```python
from build123d import *

# Parameters (mm, degrees)
SKETCH1_R                      = 40
BOSS_EXTRUDE1_DEPTH            = 20
SKETCH2_R                      = 21
CUT_EXTRUDE1_DEPTH             = 11
SKETCH3_R                      = 18
CUT_EXTRUDE2_DEPTH             = 11
CUT_EXTRUDE3_DEPTH             = 61
M6_CLEARANCE_HOLE2_D           = 6.6
M6_CLEARANCE_HOLE2_CSINK_D     = 6.65
M6_CLEARANCE_HOLE2_CSINK_ANGLE = 90


with BuildPart() as part:
    # Sketch1 → Boss-Extrude1 (new body)
    with BuildSketch(Plane(origin=(0, 0, 0), x_dir=(1, 0, 0), z_dir=(0, 1, 0))):
        with Locations(Location((0, 0, 0), (0, 0, 270))):
            Circle(SKETCH1_R)
    extrude(amount=BOSS_EXTRUDE1_DEPTH)

    # Sketch2 → Cut-Extrude1 (cut)
    with BuildSketch(Plane(origin=(0, 20, 0), x_dir=(1, 0, 0), z_dir=(0, 1, 0))):
        with Locations(Location((0, 0, 0), (0, 0, 270))):
            Circle(SKETCH2_R)
    extrude(amount=-CUT_EXTRUDE1_DEPTH, mode=Mode.SUBTRACT)

    # Sketch3 → Cut-Extrude2 (cut)
    with BuildSketch(Plane(origin=(0, 9, 0), x_dir=(1, 0, 0), z_dir=(0, 1, 0))):
        with Locations(Location((0, 0, 0), (0, 0, 270))):
            Circle(SKETCH3_R)
    extrude(amount=-CUT_EXTRUDE2_DEPTH, mode=Mode.SUBTRACT)

    # Sketch8 → Cut-Extrude3 (cut, through all)
    with BuildSketch(Plane.XZ):
        with BuildLine():
            ThreePointArc((40, 0), (37.148351242, 14.832396974), (29, 27.549954628))
            Line((29, 27.549954628), (29, -27.549954628))
            ThreePointArc((29, -27.549954628), (37.148351242, -14.832396974), (40, 0))
        make_face()
        with BuildLine():
            ThreePointArc((-29, 27.549954628), (-40, 0), (-29, -27.549954628))
            Line((-29, -27.549954628), (-29, 27.549954628))
        make_face()
    extrude(amount=-CUT_EXTRUDE3_DEPTH, mode=Mode.SUBTRACT)

    # M6 Clearance Hole2 (through all)
    with Locations(Plane(origin=(0, 0, 0), x_dir=(-1, 0, 0), z_dir=(0, -1, 0))):
        with Locations((-15, -27.5), (15, -27.5), (15, 27.5), (-15, 27.5)):
            CounterSinkHole(M6_CLEARANCE_HOLE2_D / 2, M6_CLEARANCE_HOLE2_CSINK_D / 2, counter_sink_angle=M6_CLEARANCE_HOLE2_CSINK_ANGLE)


solid = part.part
```
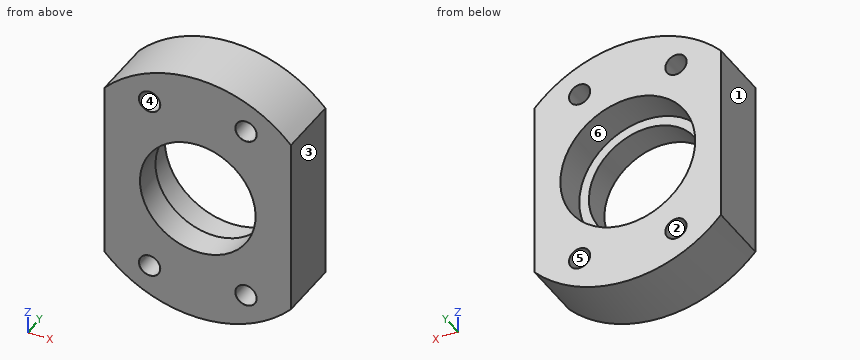
Source: CAD feature listing. Evaluate the final solid. Frame: model axes, mm. Face numbers are marked on the shaded views. A direction names the side the tool comes from. Round coordinates to 2 decimals unless told otherwise and drop trailing zeros. Order: outer loops, then holes, each group sorted by start corner. A loop starts at its lowest first (then second) coordinate and runs counter-clockwise, first axis right, second up. Notation, with made-up numbers: (77.25, 77.25) -> (86.25, 77.25) arc R24 ccw to (86.25, 92.25) -> close; hole circle Ø8 at (79, -26). An arc over 180 degrees is marked (long way). One line per item, written item: value. Start each with the question number.
Q1. Draft query along X for the marked faces 1, 2, 3 and 4. Return one class per face: pulls with the +X half, pulls with the -X half, needs draft (parallel to the pull), parting line crosses it, or undercut.
Q2. Section query C-C (y = 6.5). Return the cut outline in (x, z).
Q3. Pin query (flat end, axial travel): pin 1 (4 mm diameter, centred on x = -15, z = -27.5, fed in from +Y); pin 2 (6 mm diameter, centred on x = 17, z = 15, fed in from -Y); pin 3 (3 mm diameter, centred on x = -9.5, y = 16, fed in from -Z). Return the tip coordinate at first contact, or that it passes through.
Q4. Section query A-A (z = 0). Return the cut outline in (x, y).
Q5. Material intervals for probe 1 along X at (y, z) = (14.75, -27.5); probe 2 along Z at (x, y) = (16, 13.25); probe 3 along Z at (x, y) = (-13, 7.75), sorted ascending.
Q6. Access query for the marked faces 5 and 6. Directions: +Z, -Z, +X, -X, +Y, -Y. A direction counts if a zero-diameter tool reaches every point of the face in a straight line with its end or side. Return the directions, or none.
Q7. Section query B-B (x = 0). Return the cut outline in (y, z), plus the area to 3 significant figures.
Q8. Section query D-D (x = -15). Return the cut outline in (y, z) (3 decimals), plus the area to 3 significant figures.
Findings below:
1. face 1: pulls with the -X half
1. face 2: undercut
1. face 3: pulls with the +X half
1. face 4: undercut
2. outline: (-29, -27.55) arc R40 ccw to (29, -27.55) -> (29, 27.55) arc R40 ccw to (-29, 27.55) -> close; hole circle Ø6.6 at (-15, -27.5); hole circle Ø6.6 at (-15, 27.5); hole circle Ø36 at (0, 0); hole circle Ø6.6 at (15, -27.5); hole circle Ø6.6 at (15, 27.5)
3. pin 1: through
3. pin 2: y = 0
3. pin 3: z = -39.19
4. outline: (-29, 0) -> (-18, 0) -> (-18, 9) -> (-21, 9) -> (-21, 20) -> (-29, 20) -> close; (18, 0) -> (29, 0) -> (29, 20) -> (21, 20) -> (21, 9) -> (18, 9) -> close
5. probe 1: -29 to -18.3, -11.7 to 11.7, 18.3 to 29
5. probe 2: -36.66 to -30.64, -24.36 to -13.6, 13.6 to 24.36, 30.64 to 36.66
5. probe 3: -37.83 to -30.12, -24.88 to -12.45, 12.45 to 24.88, 30.12 to 37.83
6. face 5: +Y, -Y
6. face 6: +Y
7. outline: (0, -40) -> (20, -40) -> (20, -21) -> (9, -21) -> (9, -18) -> (0, -18) -> close; (0, 18) -> (9, 18) -> (9, 21) -> (20, 21) -> (20, 40) -> (0, 40) -> close
7. area: 814 mm²
8. outline: (0, -37.081) -> (20, -37.081) -> (20, -30.8) -> (0.025, -30.8) -> (0, -30.825) -> close; (0, -24.175) -> (0.025, -24.2) -> (20, -24.2) -> (20, -14.697) -> (9, -14.697) -> (9, -9.95) -> (0, -9.95) -> close; (0, 9.95) -> (9, 9.95) -> (9, 14.697) -> (20, 14.697) -> (20, 24.2) -> (0.025, 24.2) -> (0, 24.175) -> close; (0, 30.825) -> (0.025, 30.8) -> (20, 30.8) -> (20, 37.081) -> (0, 37.081) -> close
8. area: 717 mm²
